Here's how the part is built. I have some questions about the finished solid (model axes, mm). A direction names the side the tool comes from. Round coordinates to 2 decimals unless told otherwise and drop trailing zeros. Order: outer loops, then holes, each group sorted by start corner. A loop starts at its lowest first (then second) coordinate and runs counter-clockwise, first axis right, second up. Notation, with made-up numbers: (42, -35.5) -> (57, -35.5) arc R12 cw to (57, -22.5) -> close; hole circle Ø1 at (41, -22.75). An arc over 180 degrees is marked (long way). Use a Markdown table: item, result. Add a question column.
from build123d import *

# Parameters (mm, degrees)
SKETCH_1_W          = 115
SKETCH_1_H          = 115
SKETCH_1_R          = 6.25
EXTRUDE_1_DEPTH     = 30
SKETCH_2_R          = 40
EXTRUDE_2_DEPTH     = 15
SKETCH_22_R         = 45
EXTRUDE_4_DEPTH     = 15
SKETCH_23_W         = 6.5
SKETCH_23_H         = 5
SKETCH_24_R         = 2.5
CUT_EXTRUDE_5_DEPTH = 30
SKETCH_28_R         = 3
CUT_EXTRUDE_6_DEPTH = 25


with BuildPart() as part:
    # 草图1 → 凸台-拉伸1 (new body)
    with BuildSketch(Plane.XY):
        Rectangle(SKETCH_1_W, SKETCH_1_H)
        with Locations((-45, 45)):
            Circle(SKETCH_1_R, mode=Mode.SUBTRACT)
        with Locations((45, 45)):
            Circle(SKETCH_1_R, mode=Mode.SUBTRACT)
        with Locations((45, -45)):
            Circle(SKETCH_1_R, mode=Mode.SUBTRACT)
        with Locations((-45, -45)):
            Circle(SKETCH_1_R, mode=Mode.SUBTRACT)
    extrude(amount=EXTRUDE_1_DEPTH)

    # 草图2 → 凸台-拉伸2 (add)
    with BuildSketch(Plane.XY.offset(30)):
        Circle(SKETCH_2_R)
    extrude(amount=EXTRUDE_2_DEPTH)

    # 草图22 → 凸台-拉伸4 (add)
    with BuildSketch(Plane(origin=(0, 0, 0), x_dir=(-1, 0, 0), z_dir=(0, 0, -1))):
        Circle(SKETCH_22_R)
    extrude(amount=EXTRUDE_4_DEPTH)

    # 草图23 → 切除-旋转2 (revolve, cut)
    with BuildSketch(Plane(origin=(0, 0, 0), x_dir=(0, 0, -1), z_dir=(1, 0, 0)), mode=Mode.PRIVATE) as cut_revolve_2_sk:
        Polygon((-45, 19), (-42, 19), (-42, 21), (-36, 21), (-36, 17.5), (-29, 17.5), (-29, 18), (-25, 18), (-25, 17.5), (-18, 17.5), (-18, 18), (-14, 18), (-14, 17.5), (-8, 17.5), (-8, 18), (-1.5, 18), (-1.5, 17.5), (5.5, 17.5), (5.5, 20), (12, 20), (12, 19), (15, 19), (15, 0), (-45, 0), align=None)
        with Locations((8.25, 42.5)):
            Rectangle(SKETCH_23_W, SKETCH_23_H)
    revolve(cut_revolve_2_sk.sketch.rotate(Axis((0, 0, 45), (0, 0, -1)), 90), axis=Axis((0, 0, 45), (0, 0, -1)), mode=Mode.SUBTRACT)

    # 草图24 → 切除-拉伸5 (cut)
    with BuildSketch(Plane.XY.offset(45)):
        with Locations((0, 34.5)):
            Circle(SKETCH_24_R)
    extrude(amount=-CUT_EXTRUDE_5_DEPTH, mode=Mode.SUBTRACT)

    # 草图26 → 1/4 NPT 螺纹孔2 (revolve, cut)
    with BuildSketch(Plane(origin=(0, 57.5, 14), x_dir=(0, 0, 1), z_dir=(1, 0, 0))):
        Polygon((0, 0), (0, 20.412347279), (5.5626, 17.07), (5.5626, 10.02), (5.943676082, 10.02), (6.2436883, 0), align=None)
    revolve(axis=Axis((0, 63.85, 14), (0, -1, 0)), mode=Mode.SUBTRACT)

    # 草图28 → 切除-拉伸6 (cut)
    with BuildSketch(Plane(origin=(0, 57.5, 0), x_dir=(1, 0, 0), z_dir=(0, 1, 0))):
        with Locations(Location((0, -14, 0), (0, 0, 270))):
            Circle(SKETCH_28_R)
    extrude(amount=-CUT_EXTRUDE_6_DEPTH, mode=Mode.SUBTRACT)


solid = part.part
(1) If we mould it in two halves opening along X, with no side actions, what happens to faces 4 (the flat face through (30.2, 26.5, -5)), 5 (the cylindrical face through (-8.67, -39.05, 37.39)), 6 (the cylindrical face through (48.36, -39.73, 14.79))? For each: pulls with the +X half, pulls with the -X half, needs draft (parallel to the pull), parting line crosses it, or undercut.
(2) I want a section at C-C on z = 34. List the corners of the cut face in (x, y) for me, and give its area (3 significant figures).
(3) Please list where these lines run through material, in increasing order: probe 1 along Z at (x, y) = (-14.5, -10); probe 2 along Y at (x, z) = (-45, 18); probe 3 along Y at (x, z) = (-46.5, 21.5). Write a range as from..to.
(4) I want a section at D-D on x = 0. State how many separate pieces and enclosed holes the cut face has, and give its area (3 significant figures).
(5) I'm going to push flat-ended pins straight in: P1, Ø2, axis at x = -37, y = -23.5, coming from the +Z side; P2, Ø1.5, axis at x = -10, z = -7.5, coming from the +Y side; P3, Ø3.5, axis at x = 0, z = 14, coming from the +Y side. Where does each tip first touch, or does it pass through?
(6) On a 3-axis mill with a long thin cutter (end or side, diameter ignored), from which of +Z, -Z, +X, -X, +Y, -Y can I reach the whole of each face in a straight line? I mean faces 1 (the cylindrical face through (-20.765, -39.923, -13.226)), 2 (the flat face through (2.2, 47.48, 8.7)), 3 (the cylindrical face through (-13.267, -12.165, 26.972)). Say none if no direction works.
(7) I want a section at A-A on x = 47. List the corners of the cut face in (y, z) for me, and give its area (3 significant figures).
(8) I want a section at B-B on y = 25. List the corners of the cut face in (x, z) for me, and give its area (3 significant figures).
Output:
| question | item | result |
|---|---|---|
| 1 | face 4 | needs draft |
| 1 | face 5 | parting line crosses it |
| 1 | face 6 | undercut |
| 2 | outline | circle Ø80 at (0, 0); hole circle Ø35 at (0, 0); hole circle Ø5 at (0, 34.5) |
| 2 | area | 4,040 mm² |
| 3 | probe 1 | -5.5..1.5, 8..14, 18..25, 29..36 |
| 3 | probe 2 | -57.5..-51.25, -38.75..38.75, 51.25..57.5 |
| 3 | probe 3 | -57.5..-51.07, -38.93..38.93, 51.07..57.5 |
| 4 | separate pieces | 3 |
| 4 | enclosed holes | 0 |
| 4 | area | 3,330 mm² |
| 5 | P1 | z = 30 |
| 5 | P2 | y = 38.92 |
| 5 | P3 | y = 32.5 |
| 6 | face 1 | -Z |
| 6 | face 2 | +Y |
| 6 | face 3 | none |
| 7 | outline | (-57.5, 0) -> (-50.92, 0) -> (-50.92, 30) -> (-57.5, 30) -> close; (-39.08, 0) -> (39.08, 0) -> (39.08, 30) -> (-39.08, 30) -> close; (50.92, 0) -> (57.5, 0) -> (57.5, 30) -> (50.92, 30) -> close |
| 7 | area | 2,740 mm² |
| 8 | outline | (-57.5, 0) -> (-37.42, 0) -> (-37.42, -5) -> (-31.22, -5) -> (-31.22, -11.5) -> (-37.42, -11.5) -> (-37.42, -15) -> (37.42, -15) -> (37.42, -11.5) -> (31.22, -11.5) -> (31.22, -5) -> (37.42, -5) -> (37.42, 0) -> (57.5, 0) -> (57.5, 30) -> (31.22, 30) -> (31.22, 45) -> (-31.22, 45) -> (-31.22, 30) -> (-57.5, 30) -> close |
| 8 | area | 5,430 mm² |
